```python
from build123d import *

# Parameters (mm, degrees)
SKETCH_1_W                   = 65
SKETCH_1_H                   = 120
EXTRUDE_1_DEPTH              = 12
HOLE_WIZARD_M6_1_D           = 6.6
SKETCH_4_W                   = 65
SKETCH_4_H                   = 10.1
CUT_EXTRUDE_1_DEPTH          = 2
CHAMFER_1_SIZE               = 2
HOLE_WIZARD_M4_1_D           = 4.5
HOLE_WIZARD_M4_1_CBORE_D     = 8
HOLE_WIZARD_M4_1_CBORE_DEPTH = 4.6


with BuildPart() as part:
    # 草图1 → 凸台-拉伸1 (new body)
    with BuildSketch(Plane(origin=(0, 0, 0), x_dir=(1, 0, 0), z_dir=(0, 1, 0))):
        Rectangle(SKETCH_1_W, SKETCH_1_H)
    extrude(amount=EXTRUDE_1_DEPTH)

    # M6 间隙孔1 (through all)
    with Locations(Plane(origin=(0, 12, 0), x_dir=(1, 0, 0), z_dir=(0, 1, 0))):
        with Locations((-20, -54), (20, -54), (-20, 0), (20, 0), (-20, 54), (20, 54)):
            Hole(HOLE_WIZARD_M6_1_D / 2)

    # 草图4 → 切除-拉伸1 (cut)
    with BuildSketch(Plane(origin=(0, 12, 0), x_dir=(1, 0, 0), z_dir=(0, 1, 0))):
        with Locations((0, 42.5)):
            Rectangle(SKETCH_4_W, SKETCH_4_H)
        with Locations((0, -42.5)):
            Rectangle(SKETCH_4_W, SKETCH_4_H)
    extrude(amount=-CUT_EXTRUDE_1_DEPTH, mode=Mode.SUBTRACT)

    # 倒角1
    chamfer_1_edges = [part.edges().sort_by_distance(p)[0] for p in [
        (32.5, 6, 60),
        (-32.5, 6, 60),
        (-32.5, 6, -60),
        (32.5, 6, -60),
    ]]
    chamfer(chamfer_1_edges, length=CHAMFER_1_SIZE)

    # M4 六角圆柱头螺钉的柱形沉头孔1 (through all)
    with Locations(Plane(origin=(0, 0, 0), x_dir=(-1, 0, 0), z_dir=(0, -1, 0))):
        with Locations((-25, 42.5), (-25, -42.5), (25, -42.5), (25, 42.5)):
            CounterBoreHole(HOLE_WIZARD_M4_1_D / 2, HOLE_WIZARD_M4_1_CBORE_D / 2, HOLE_WIZARD_M4_1_CBORE_DEPTH)


solid = part.part
```
The listing builds one solid part. Answer for the finished solid, in the listing's coordinates (mm). A direction names the side the tool comes from. Give positions to 0.01 mm unless a question says otherwise; leave off trailing zeros. Write each loop counter-clockwise with the first axis right and the second up, starting at its lowest first coordinate (ties: lowest second). Pieces come first, ordered by that corner, then holes. Notation, with made-up numbers: (43, 60) -> (100, 60) arc R32 ccw to (100, 89) -> close; hole circle Ø5 at (-38.75, 76). An arc over 180 degrees is marked (long way). Use one line per item in the form item = value.
1) Section D-D on x = 13.5 is taken. Write down the section's boundary in (y, z), plus the area to 3 significant figures.
Result:
outline = (0, -60) -> (12, -60) -> (12, -47.55) -> (10, -47.55) -> (10, -37.45) -> (12, -37.45) -> (12, 37.45) -> (10, 37.45) -> (10, 47.55) -> (12, 47.55) -> (12, 60) -> (0, 60) -> close
area = 1,400 mm²
2) Section B-B on z = 54 is taken. Write down the section's boundary in (x, y), plus the area to 3 significant figures.
Result:
outline = (-32.5, 0) -> (-23.3, 0) -> (-23.3, 12) -> (-32.5, 12) -> close; (-16.7, 0) -> (16.7, 0) -> (16.7, 12) -> (-16.7, 12) -> close; (23.3, 0) -> (32.5, 0) -> (32.5, 12) -> (23.3, 12) -> close
area = 622 mm²
3) Straight lines are drawn through the part: probe 1 along X at (y, z) = (5.75, 54); probe 2 along X at (y, z) = (7.45, -42.5); probe 3 along Z at (x, y) = (-20, 3). For each, find the intervals that lie inside material, in ascending order.
Result:
probe_1 = -32.5 to -23.3, -16.7 to 16.7, 23.3 to 32.5
probe_2 = -32.5 to -27.25, -22.75 to 22.75, 27.25 to 32.5
probe_3 = -60 to -57.3, -50.7 to -3.3, 3.3 to 50.7, 57.3 to 60
4) Section A-A on x = 25 is taken. Write down the section's boundary in (y, z), plus the area to 3 significant figures.
Result:
outline = (0, -60) -> (12, -60) -> (12, -47.55) -> (10, -47.55) -> (10, -44.75) -> (4.6, -44.75) -> (4.6, -46.5) -> (0, -46.5) -> close; (0, -38.5) -> (4.6, -38.5) -> (4.6, -40.25) -> (10, -40.25) -> (10, -37.45) -> (12, -37.45) -> (12, 37.45) -> (10, 37.45) -> (10, 40.25) -> (4.6, 40.25) -> (4.6, 38.5) -> (0, 38.5) -> close; (0, 46.5) -> (4.6, 46.5) -> (4.6, 44.75) -> (10, 44.75) -> (10, 47.55) -> (12, 47.55) -> (12, 60) -> (0, 60) -> close
area = 1,280 mm²
5) Each of these flat-tipped pins is pushed along its axis until it touches: P1, Ø4, axis at x = 25, z = -41, coming from the -Y side; P2, Ø6, axis at x = -25, z = 42.5, coming from the +Y side. Where does it stop, or does it pass through?
Result:
P1 = 4.6
P2 = 10
6) For a pull along Z with two mould halves and no side action, classify faces 1 (the flat face through (0, 0, -1)), 2 (the cylindrical face through (26.21, 7.338, 40.603)) as +Z half, -Z half, draft (parallel to the pull), parting line (faces both ways), or undercut.
Result:
face_1 = draft
face_2 = undercut
7) A tool of negligible diameter and unlimited length cuts with its end or side. For faces 3 (the cylindrical face through (-19.57, 5.92, 50.73)), 4 (the flat face through (23, 4.6, -41)), 5 (the flat face through (0, 10, 42)), from which of +Z, -Z, +X, -X, +Y, -Y can it reach the whole face along a straight path? Write none if from no direction.
Result:
face_3 = +Y, -Y
face_4 = -Y
face_5 = +X, -X, +Y
8) Section C-C on y = 8.75 is taken. Count the separate pieces of the cut face and the enclosed holes in it, plus the area to 3 significant figures.
Result:
separate_pieces = 1
enclosed_holes = 10
area = 7,520 mm²
